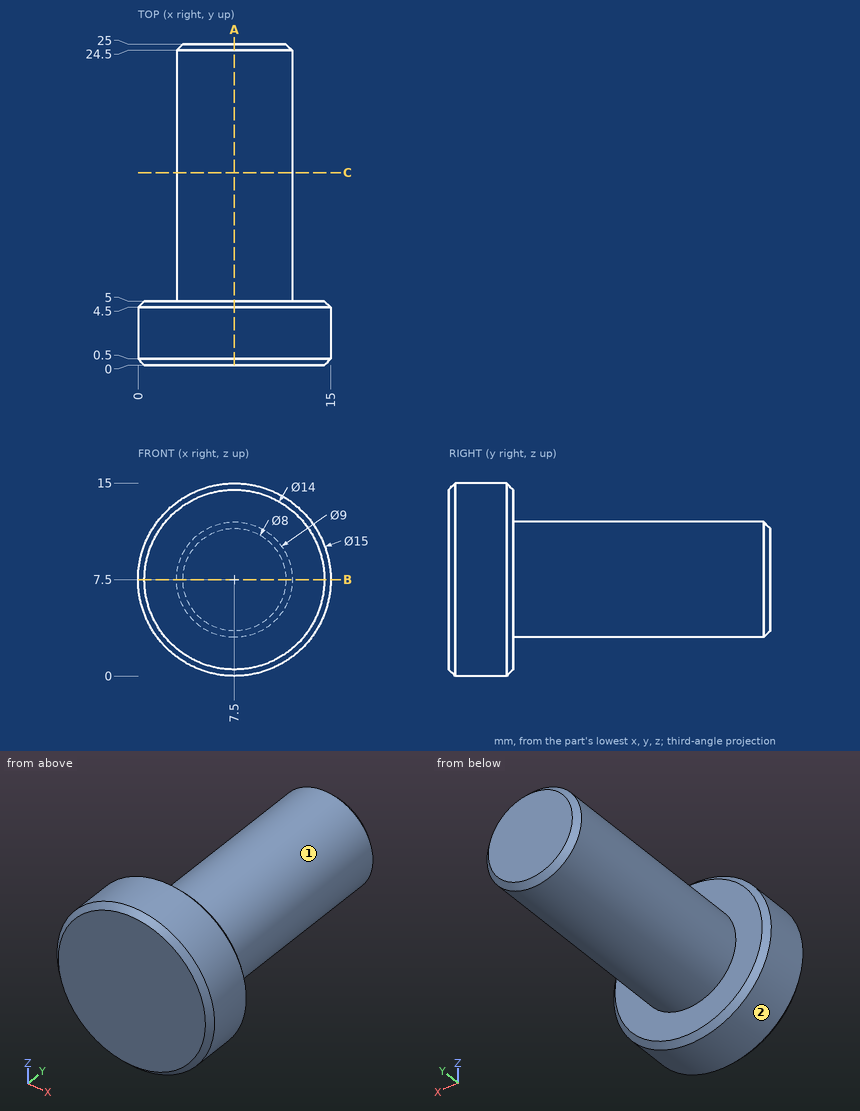
Source: three-view drawing plus pictorial views. Frame: mm from the lowest corner of the part. A direction names the side the tool comes from. Round coordinates to 2 decimals unless told otherwise and drop trailing zeros. Loops run counter-clockwise (first coordinate to the right, second up) from the corner with the lowest first, then second, coordinate; pieces in that order, holes last. Notation, with made-up numbers: (-6, 6.5) -> (53, 6.5) arc R9 cw to (53, 20.5) -> close; hole circle Ø1 at (-38.5, 59). An arc over 180 degrees is marked (long way). Use one line per item in the form item = value.
Item 1: Access query for the marked faces 1 and 2. Directions: +Z, -Z, +X, -X, +Y, -Y. A direction counts if a zero-diameter tool reaches every point of the face in a straight line with its end or side. Return the directions, or none.
Evaluation:
face_1 = +Y
face_2 = +Y, -Y
Item 2: Cut plane B-B on z = 7.5. Output: boundary loops of the cut face in (x, y).
Evaluation:
outline = (0, 0.5) -> (0.5, 0) -> (14.5, 0) -> (15, 0.5) -> (15, 4.5) -> (14.5, 5) -> (12, 5) -> (12, 24.5) -> (11.5, 25) -> (3.5, 25) -> (3, 24.5) -> (3, 5) -> (0.5, 5) -> (0, 4.5) -> close
Item 3: Cut plane C-C on y = 15. Output: boundary loops of the cut face in (x, z).
Evaluation:
outline = circle Ø9 at (7.5, 7.5)
Item 4: Contact query for flat-ended pins moving along their axis: pin 1 Ø1.5 at (x, y) = (7, 6) entering from +Z; pin 2 Ø3 at (x, y) = (3, 18.5) entering from -Z; pin 3 Ø4 at (y, z) = (21, 2.5) entering from -X. Output: stop coordinate, or through.
Evaluation:
pin_1 = 12
pin_2 = 4.15
pin_3 = 4.15
Item 5: Cut plane A-A on x = 7.5. Output: boundary loops of the cut face in (y, z).
Evaluation:
outline = (0, 0.5) -> (0.5, 0) -> (4.5, 0) -> (5, 0.5) -> (5, 3) -> (24.5, 3) -> (25, 3.5) -> (25, 11.5) -> (24.5, 12) -> (5, 12) -> (5, 14.5) -> (4.5, 15) -> (0.5, 15) -> (0, 14.5) -> close
Item 6: Material intervals for probe 1 along Y at (x, z) = (11.75, 3.25); probe 2 along Z at (x, y) = (7.5, 9.5); probe 3 along X at (y, z) = (13.75, 10.25), sorted ascending.
Evaluation:
probe_1 = 0 to 5
probe_2 = 3 to 12
probe_3 = 3.94 to 11.06
